Geometry check sheet. Reference: the model listing, model coordinates, mm. A direction names the side the tool comes from. Round coordinates to 2 decimals unless told otherwise and drop trailing zeros. Order: outer loops, then holes, each group sorted by start corner. A loop starts at its lowest first (then second) coordinate and runs counter-clockwise, first axis right, second up. Notation, with made-up numbers: (53.5, 53) - (104.5, 53) arc R6 ccw to (104.5, 64) - close; hole circle Ø1 at (46.5, 87.25). An arc over 180 degrees is marked (long way). One line per question, with ' | ' between items. Start each with the question number.
Q1. Material ranges on line 1 along Z through (x, y) = (1.5, 0.75); line 2 along Y through (x, z) = (5.5, 0); line 3 along Y through (x, z) = (1, -0.5), recorded low to high.
Q2. Tool access check on faces 5 (the face through (2.226, 3.905, -0.867)), 6 (the face through (3.1, 2, -2)), 7 (the face through (0.928, 0.215, 0.762)). Record the directions out of +Z, -Z, +X, -X, +Y, -Y that give a thin tool (end or side, any length) a straight path to the whole face; none if there is none.
Q3. Sectioned sample at C-C, the plane x = 9.5. Enter the section's corners in (y, z), then the cut area to 3 significant figures.
Q4. Gauge pin test, flat ends, axial feed: P1, Ø1.5, axis at x = 8.5, y = -2, coming from the +Z side; P2, Ø4, axis at x = 10, y = -3, coming from the -Z side; P3, Ø2, axis at x = 5, z = -1.5, coming from the +Y side. Record the tip position at first contact, or that the pin passes through.
Q5. Sectioned sample at A-A, the plane x = 2. Enter the section's corners in (y, z).
Q6. Sectioned sample at D-D, the plane z = 2.75. Enter the section's corners in (x, y), then the cut area to 3 significant figures.
Q7. Sectioned sample at B-B, the plane y = -2.5. Enter the section's corners in (x, z), then the cut area to 3 significant figures.
Q8. Mould release check, pull along X, two halves, no side actions. Record for faces 1 (the face through (8, 2, 0)), 2 (the face through (3.97, -0.52, 1.65)), 3 (the face through (11.1, 0, 0)), 4 (the face through (0.928, 0.735, -0.215)): +X half, -X half, draft (parallel to the pull), parting line (faces both ways), or undercut.
```python
from build123d import *


with BuildPart() as part:
    # Sketch2 → Base-Revolve (revolve)
    with BuildSketch(Plane.XY, mode=Mode.PRIVATE) as base_revolve_sk:
        with BuildLine():
            Line((0, 0), (11.1, 0))
            Line((11.1, 0), (11.1, 2))
            Line((11.1, 2), (4.5, 2))
            Line((4.5, 2), (4.232, 1.732))
            Line((4.232, 1.732), (3.718, 1.732))
            ThreePointArc((3.718, 1.732), (3.281008009, 1.913008009), (3.1, 2.35))
            Line((3.1, 2.35), (3.1, 4))
            Line((3.1, 4), (1.376524617, 4))
            ThreePointArc((1.376524617, 4), (0.353757652, 2.115113473), (0, 0))
        make_face()
    revolve(base_revolve_sk.sketch.rotate(Axis((-1.331757704, 0, 0), (1, 0, 0)), 90), axis=Axis((-1.331757704, 0, 0), (1, 0, 0)))

    # Sketch3 → Cut-Revolve1 (revolve, cut)
    with BuildSketch(Plane.XY, mode=Mode.PRIVATE) as cut_revolve1_sk:
        Polygon((10.753791204, 2), (11.453791204, 2), (11.1, 1.3938), align=None)
    revolve(cut_revolve1_sk.sketch.rotate(Axis((-0.242766179, 0, 0), (1, 0, 0)), 90), axis=Axis((-0.242766179, 0, 0), (1, 0, 0)), mode=Mode.SUBTRACT)

    # Sketch5 → Cut-Loft1 section 0
    with BuildSketch(Plane(origin=(0, 0, 0), x_dir=(0, 0, -1), z_dir=(1, 0, 0)), mode=Mode.PRIVATE) as cut_loft1_s0:
        with BuildLine():
            Line((0.35, 2.2), (-0.35, 2.2))
            Line((-0.35, 2.2), (-0.35, -2.2))
            Line((-0.35, -2.2), (0.35, -2.2))
            Line((0.35, -2.2), (0.35, 2.2))
        make_face()
    cut_loft1 = loft([Vertex(2.4, 0, 0), cut_loft1_s0.sketch], mode=Mode.SUBTRACT)

    # Mirror1: Cut-Loft1 across plane
    add(cut_loft1.mirror(Plane(origin=(0, 0, 0), x_dir=(0, 0.7071067811865462, 0.7071067811865488), z_dir=(0, -0.7071067811865488, 0.7071067811865462))), mode=Mode.SUBTRACT)


solid = part.part
```
Determined:
1) line 1: z = -3.93 to -0.13, 0.13 to 3.93 | line 2: y = -2 to 2 | line 3: y = -3.43 to -0.2, 0.2 to 3.43
2) face 5: +X, -X | face 6: +X | face 7: -X
3) outline: circle Ø4 at (0, 0) | area: 12.6 mm2
4) P1: stops at z = 1.56 | P2: stops at z = -1.73 | P3: stops at y = 1.94
5) outline: circle Ø8 at (0, 0); hole (-0.37, -0.06) - (-0.06, -0.06) - (-0.06, -0.37) - (0.06, -0.37) - (0.06, -0.06) - (0.37, -0.06) - (0.37, 0.06) - (0.06, 0.06) - (0.06, 0.37) - (-0.06, 0.37) - (-0.06, 0.06) - (-0.37, 0.06) - close
6) outline: (1.38, -2.9) - (3.1, -2.9) - (3.1, 2.9) - (1.38, 2.9) arc R5.89 ccw to start | area: 13.0 mm2
7) outline: (1.38, -3.12) - (3.1, -3.12) - (3.1, 3.12) - (1.38, 3.12) arc R6 ccw to start | area: 14.5 mm2
8) face 1: draft | face 2: undercut | face 3: +X half | face 4: -X half
